Design review of the part built by this model. Coordinates are the model's own, in mm. A direction names the side the tool comes from. Coordinates: 2 decimals unless noted, no trailing zeros. Loops run counter-clockwise (first coordinate to the right, second up) from the corner with the lowest first, then second, coordinate; pieces in that order, holes last. Notation, with made-up numbers: (42, 0) - (68, 0) arc R15 ccw to (68, 4) - close; hole circle Ø6 at (-2.5, -27.75). An arc over 180 degrees is marked (long way). Answer in a Markdown table with one row per item. Add a question column.
(1) We need section B-B, the plane y = -110. Write out the cut boundary in (x, z).
(2) Clearance check with flat-ended pins moving along their axes: pin 1 (6 mm diameter, centred on x = 27, y = -106, fed in from +Z); pin 2 (10 mm diameter, centred on x = -58, z = -20, fed in from -Y); pin 3 (13 mm diameter, centred on y = -54, z = 3, fed in from -X). State where each tip first meets the part, or that it passes through.
(3) For faces 1 (the face through (1, 6, 45)), 2 (the face through (0, 8, 164)), 3 (the face through (28.796, -73, 0)), list the 3-axis set-ups (+Z, -Z, +X, -X, +Y, -Y) from which the entire face can be reached by the end or side of a thin tool; tool diameter is ignored.
(4) We need section D-D, the plane z = 140. Write out the cut boundary in (x, y).
(5) To check wall thickness, follow L1, parallel to X at y = -60, z = 2; L2, parallel to Y at x = -92.5, z = 18; L3, parallel to Z at x = -18.5, y = -142.5. State the ranges of each line that lie inside material, in increasing order. Write a range as [from, to].
(6) The part is to be moulded in two halves that separate along Z. For faces 4 (the face through (-74.265, 7.888, 72.439)), 5 (the face through (-18, 16, 18)), 6 (the face through (12.62, 11.07, 40.06)), say which applies: released by +Z, released by -Z, zero draft, split by the parting line, or undercut.
(7) We need section C-C, the plane x = 0. Give the number of separate pieces and of enclosed holes in the cut face, plus the area to 3 significant figures.
(8) We need section A-A, the plane z = 0. Write out the cut boundary in (x, y), plus the area to 3 significant figures.
from build123d import *

# Parameters (mm, degrees)
SQUARE_FLANGE_PROFILE_SKETCH_R = 12
SQUARE_FLANGE_240X16_DEPTH     = 16
FLANGE_STEP_CIRCLE_SKETCH_R    = 103.5
FLANGE_STEP_CUT_207_DEPTH      = 10
ARC_SLOTS_R78_DEPTH            = 60
HUB_SKETCH_R                   = 42
HUB_84_DEPTH                   = 180
BORE_SKETCH_R                  = 24
BORE_48_DEPTH                  = 180
KEYWAY_SKETCH_W                = 5.55
KEYWAY_SKETCH_H                = 11.94
KEYWAY_DEPTH                   = 180


with BuildPart() as part:
    # Square Flange Profile Sketch → Square Flange 240x16 (new body)
    with BuildSketch(Plane(origin=(0, 0, 0), x_dir=(1, 0, 0), z_dir=(0, 1, 0))):
        with BuildLine():
            ThreePointArc((22.095900417, 149.368627689), (0, 164), (-22.095900417, 149.368627689))
            ThreePointArc((-22.095900417, 149.368627689), (-73.349277098, 73.349277098), (-149.368627689, 22.095900417))
            ThreePointArc((-149.368627689, 22.095900417), (-164, 0), (-149.368627689, -22.095900417))
            ThreePointArc((-149.368627689, -22.095900417), (-73.349277098, -73.349277098), (-22.095900417, -149.368627689))
            ThreePointArc((-22.095900417, -149.368627689), (0, -164), (22.095900417, -149.368627689))
            ThreePointArc((22.095900417, -149.368627689), (73.349277098, -73.349277098), (149.368627689, -22.095900417))
            ThreePointArc((149.368627689, -22.095900417), (164, 0), (149.368627689, 22.095900417))
            ThreePointArc((149.368627689, 22.095900417), (73.349277098, 73.349277098), (22.095900417, 149.368627689))
        make_face()
        with Locations(Location((0, 140, 0), (0, 0, 270))):
            Circle(SQUARE_FLANGE_PROFILE_SKETCH_R, mode=Mode.SUBTRACT)
        with Locations(Location((140, 0, 0), (0, 0, 270))):
            Circle(SQUARE_FLANGE_PROFILE_SKETCH_R, mode=Mode.SUBTRACT)
        with Locations(Location((0, -140, 0), (0, 0, 270))):
            Circle(SQUARE_FLANGE_PROFILE_SKETCH_R, mode=Mode.SUBTRACT)
        with Locations(Location((-140, 0, 0), (0, 0, 270))):
            Circle(SQUARE_FLANGE_PROFILE_SKETCH_R, mode=Mode.SUBTRACT)
    extrude(amount=SQUARE_FLANGE_240X16_DEPTH)

    # Flange Step Circle Sketch → Flange Step Cut Ø207 (cut)
    with BuildSketch(Plane(origin=(0, 16, 0), x_dir=(1, 0, 0), z_dir=(0, 1, 0))):
        with Locations(Location((0, 0, 0), (0, 0, 270))):
            Circle(FLANGE_STEP_CIRCLE_SKETCH_R)
    extrude(amount=-FLANGE_STEP_CUT_207_DEPTH, mode=Mode.SUBTRACT)

    # Arc Slots Sketch → Arc Slots R78 (cut)
    with BuildSketch(Plane(origin=(0, 6, 0), x_dir=(1, 0, 0), z_dir=(0, 1, 0))):
        with BuildLine():
            ThreePointArc((55.154328933, 55.154328933), (0, 78), (-55.154328933, 55.154328933))
            ThreePointArc((-55.154328933, 55.154328933), (-55.154328933, 42.426406871), (-42.426406871, 42.426406871))
            ThreePointArc((-42.426406871, 42.426406871), (0, 60), (42.426406871, 42.426406871))
            ThreePointArc((42.426406871, 42.426406871), (55.154328933, 42.426406871), (55.154328933, 55.154328933))
        make_face()
        with BuildLine():
            ThreePointArc((42.426406871, -42.426406871), (0, -60), (-42.426406871, -42.426406871))
            ThreePointArc((-42.426406871, -42.426406871), (-55.154328933, -42.426406871), (-55.154328933, -55.154328933))
            ThreePointArc((-55.154328933, -55.154328933), (0, -78), (55.154328933, -55.154328933))
            ThreePointArc((55.154328933, -55.154328933), (55.154328933, -42.426406871), (42.426406871, -42.426406871))
        make_face()
    extrude(amount=-ARC_SLOTS_R78_DEPTH, mode=Mode.SUBTRACT)

    # Hub Sketch → Hub Ø84 (add)
    with BuildSketch(Plane(origin=(0, 16, 0), x_dir=(1, 0, 0), z_dir=(0, 1, 0))):
        with Locations(Location((0, 0, 0), (0, 0, 270))):
            Circle(HUB_SKETCH_R)
    extrude(amount=-HUB_84_DEPTH)

    # Bore Sketch → Bore Ø48 (cut)
    with BuildSketch(Plane(origin=(0, 16, 0), x_dir=(1, 0, 0), z_dir=(0, 1, 0))):
        with Locations(Location((0, 0, 0), (0, 0, 270))):
            Circle(BORE_SKETCH_R)
    extrude(amount=-BORE_48_DEPTH, mode=Mode.SUBTRACT)

    # Keyway Sketch → Keyway (cut)
    with BuildSketch(Plane(origin=(0, 16, 0), x_dir=(1, 0, 0), z_dir=(0, 1, 0))):
        with Locations((26.020625395, 0)):
            Rectangle(KEYWAY_SKETCH_W, KEYWAY_SKETCH_H)
    extrude(amount=-KEYWAY_DEPTH, mode=Mode.SUBTRACT)


solid = part.part
Responses:
| question | item | result |
|---|---|---|
| 1 | outline | circle Ø84 at (0, 0); hole (23.25, -5.97) - (28.8, -5.97) - (28.8, 5.97) - (23.25, 5.97) arc R24 ccw (long way) to start |
| 2 | pin 1 | stops at z = 34.47 |
| 2 | pin 2 | stops at y = 0 |
| 2 | pin 3 | stops at x = -42 |
| 3 | face 1 | +Y |
| 3 | face 2 | +Z, +Y, -Y |
| 3 | face 3 | +Y, -Y |
| 4 | outline | (-26.31, 0) - (-12, 0) - (-12, 16) - (-26.31, 16) - close; (12, 0) - (26.31, 0) - (26.31, 16) - (12, 16) - close |
| 5 | L1 | x = [-41.95, -23.92], [28.8, 41.95] |
| 5 | L2 | y = [0, 6] |
| 5 | L3 | z = [-37.71, -15.29], [15.29, 37.71] |
| 6 | face 4 | released by +Z |
| 6 | face 5 | zero draft |
| 6 | face 6 | undercut |
| 7 | separate pieces | 6 |
| 7 | enclosed holes | 0 |
| 7 | area | 8,170 mm2 |
| 8 | outline | (-164, 0) - (-152, 0) - (-152, 16) - (-164, 16) - close; (-128, 0) - (-42, 0) - (-42, -164) - (-24, -164) - (-24, 16) - (-42, 16) - (-42, 6) - (-103.5, 6) - (-103.5, 16) - (-128, 16) - close; (28.8, -164) - (42, -164) - (42, 0) - (128, 0) - (128, 16) - (103.5, 16) - (103.5, 6) - (42, 6) - (42, 16) - (28.8, 16) - close; (152, 0) - (164, 0) - (164, 16) - (152, 16) - close |
| 8 | area | 7,520 mm2 |
